from build123d import *

# Parameters (mm, degrees)
COLLAR_BODY_SKETCH_R   = 25
COLLAR_BODY_DEPTH      = 15
COLLAR_BODY_SKETCH_R_2 = 8
COLLAR_BODY_2_DEPTH    = 15
COLLAR_BODY_SKETCH_R_3 = 10
COLLAR_BODY_3_DEPTH    = 15
LINK_LUGS_DEPTH        = 5
CLAMP_SLOT_SKETCH_R    = 20
CLAMP_SLOT_SKETCH_R_2  = 4
CLAMP_SLOT_CUT_DEPTH   = 77.215631599


with BuildPart() as part:
    # Collar Body Sketch → Collar Body (new, symmetric)
    with BuildSketch(Plane.XY):
        Circle(COLLAR_BODY_SKETCH_R)
    extrude(amount=COLLAR_BODY_DEPTH, both=True)



with BuildPart() as body_2:
    # Collar Body Sketch → Collar Body 2 (new, symmetric)
    with BuildSketch(Plane.XY):
        with Locations((-50, 0)):
            Circle(COLLAR_BODY_SKETCH_R_2)
    extrude(amount=COLLAR_BODY_2_DEPTH, both=True)


with BuildPart() as body_3:
    # Collar Body Sketch → Collar Body 3 (new, symmetric)
    with BuildSketch(Plane.XY):
        with Locations((40, 0)):
            Circle(COLLAR_BODY_SKETCH_R_3)
    extrude(amount=COLLAR_BODY_3_DEPTH, both=True)


with BuildPart() as part_1:
    add(part.part)

    add(body_2.part)  # Link Lugs merges body 2

    add(body_3.part)  # Link Lugs merges body 3
    # Link Lugs Sketch → Link Lugs (add, symmetric)
    with BuildSketch(Plane.XY):
        with BuildLine():
            Line((-65, -5.297031987), (-65, 5.297031987))
            ThreePointArc((-65, 5.297031987), (-62.656854249, 10.953886237), (-57, 13.297031987))
            Line((-57, 13.297031987), (-36, 13.297031987))
            ThreePointArc((-36, 13.297031987), (-19.718668513, 24.43538565), (0, 25))
            ThreePointArc((0, 25), (4.775431561, 24.539666937), (9.375, 23.175620272))
            Line((9.375, 23.175620272), (43.75, 9.270248109))
            ThreePointArc((43.75, 9.270248109), (50, 0), (43.75, -9.270248109))
            Line((43.75, -9.270248109), (9.375, -23.175620272))
            ThreePointArc((9.375, -23.175620272), (4.775431561, -24.539666937), (0, -25))
            ThreePointArc((0, -25), (-19.718668513, -24.43538565), (-36, -13.297031987))
            Line((-36, -13.297031987), (-57, -13.297031987))
            ThreePointArc((-57, -13.297031987), (-62.656854249, -10.953886237), (-65, -5.297031987))
        make_face()
    extrude(amount=LINK_LUGS_DEPTH, both=True)

    # Clamp Slot Sketch → Clamp Slot Cut (cut, through all)
    with BuildSketch(Plane.XY.offset(15)):
        Circle(CLAMP_SLOT_SKETCH_R)
        with Locations((-50, 0)):
            Circle(CLAMP_SLOT_SKETCH_R_2)
        with BuildLine():
            Line((40.845051729, 2), (40.845051729, -2))
            Line((40.845051729, -2), (49.145051729, -2))
            Line((49.145051729, -2), (49.638757615, -2.663522411))
            ThreePointArc((49.638757615, -2.663522411), (50, 0), (49.638757615, 2.663522411))
            Line((49.638757615, 2.663522411), (49.138757615, 2))
            Line((49.138757615, 2), (40.845051729, 2))
        make_face()
    extrude(amount=-CLAMP_SLOT_CUT_DEPTH, mode=Mode.SUBTRACT)


solid = part_1.part
Model file for the job. Use its own axes, mm. A direction names the side the tool comes from. Coordinates: 2 decimals unless noted, no trailing zeros. Loops run counter-clockwise (first coordinate to the right, second up) from the corner with the lowest first, then second, coordinate; pieces in that order, holes last. Notation, with made-up numbers: (-32.5, -9) -> (2.5, -9) arc R19 ccw to (2.5, 28) -> close; hole circle Ø5 at (27, -13.75). An arc over 180 degrees is marked (long way). Use one line per item in the form item = value. Start each with the question number.
(1) Tool access for faces 1 (the flat face through (-46, -13.297, 0)), 2 (the flat face through (-39, 0, 5)), 3 (the flat face through (45, 2, 0)), 4 (the flat face through (-47, 13.297, 0)): list every direction of +Z, -Z, +X, -X, +Y, -Y with a clear straight run to the whole face (end or side of a thin tool).
(2) Flat gauge pins, fed straight in: pin 1 (3 mm diameter, centred on y = 13.5, z = -11.5, fed in from -X); pin 2 (3 mm diameter, centred on x = -45.5, y = -11, fed in from +Z); pin 3 (5 mm diameter, centred on x = -51.5, z = 2, fed in from +Y). Where does each tip first touch, or does it go through?
(3) Cut at C-C on x = -50. Give the cut face in (y, z).
(4) Probe probe 1 along Y at (x, z) = (-1, -6); probe 2 along Y at (x, z) = (-50, 4); probe 3 along X at (y, z) = (14, -9). List the from-to ranges inside material, lowest first. Write a range as from..to.
(5) Cut at B-B on y = 0. Give the number of separate pieces and of enclosed holes in the cut face, and give its area (3 significant figures).
(6) Cut at D-D on z = 1. Give the cut face in (x, y) (3 decimals), and give its area (3 significant figures).
(7) Cut at A-A on z = 8. Give the cut face in (x, y), and give its area (3 significant figures).
(8) Pull direction Y, two halves, no side cores. Call faces 5 (the cylindrical face through (-62.59, -11.02, 0.07)), 6 (the flat face through (45, -2, 0)), 7 (the flat face through (-39, 0, -5)), 8 (the cylindrical face through (-4.336, -19.524, 0.21)): pulls with the +Y half, pulls with the -Y half, needs draft (parallel to the pull), parting line crosses it, or undercut.
Values:
q1.face_1 = +Z, -Z, -X, -Y
q1.face_2 = +Z
q1.face_3 = +Z, -Z, +X
q1.face_4 = +Z, -Z, -X, +Y
q2.pin_1 = -21.93
q2.pin_2 = 5
q2.pin_3 = 13.3
q3.outline = (-13.3, -5) -> (-8, -5) -> (-8, -15) -> (-4, -15) -> (-4, 15) -> (-8, 15) -> (-8, 5) -> (-13.3, 5) -> close; (4, -15) -> (8, -15) -> (8, -5) -> (13.3, -5) -> (13.3, 5) -> (8, 5) -> (8, 15) -> (4, 15) -> close
q4.probe_1 = -24.98..-19.97, 19.97..24.98
q4.probe_2 = -13.3..-4, 4..13.3
q4.probe_3 = -20.71..-14.28, 14.28..20.71
q5.separate_pieces = 3
q5.enclosed_holes = 0
q5.area = 1,160 mm2
q6.outline = (-65, -5.297) arc R8 ccw to (-57, -13.297) -> (-36, -13.297) arc R35 ccw to (0, -25) arc R25 ccw to (9.375, -23.176) -> (43.75, -9.27) arc R10 ccw to (49.639, -2.664) -> (49.145, -2) -> (40.845, -2) -> (40.845, 2) -> (49.139, 2) -> (49.639, 2.664) arc R10 ccw to (43.75, 9.27) -> (9.375, 23.176) arc R25 ccw to (0, 25) arc R35 ccw to (-36, 13.297) -> (-57, 13.297) arc R8 ccw to (-65, 5.297) -> close; hole circle Ø8 at (-50, 0); hole circle Ø40 at (0, 0)
q6.area = 2,720 mm2
q7.outline = circle Ø16 at (-50, 0); circle Ø50 at (0, 0); (40.85, -2) -> (40.85, 2) -> (49.14, 2) -> (49.64, 2.66) arc R10 ccw (long way) to (49.64, -2.66) -> (49.15, -2) -> close; hole circle Ø8 at (-50, 0); hole circle Ø40 at (0, 0)
q7.area = 1,140 mm2
q8.face_5 = pulls with the -Y half
q8.face_6 = undercut
q8.face_7 = needs draft
q8.face_8 = undercut
